from build123d import *

# Parameters (mm, degrees)
SKETCH1_R           = 1.5
BOSS_EXTRUDE1_DEPTH = 3


with BuildPart() as part:
    # Sketch1 → Boss-Extrude1 (new body)
    with BuildSketch(Plane(origin=(0, 0, 0), x_dir=(1, 0, 0), z_dir=(0, 1, 0))):
        with BuildLine():
            Line((0, 2.5), (13, 2.5))
            ThreePointArc((13, 2.5), (15.5, 0), (13, -2.5))
            Line((13, -2.5), (0, -2.5))
            ThreePointArc((0, -2.5), (-2.5, 0), (0, 2.5))
        make_face()
        with Locations(Location((0, 0, 0), (0, 0, 270))):
            Circle(SKETCH1_R, mode=Mode.SUBTRACT)
        with Locations(Location((13, 0, 0), (0, 0, 270))):
            Circle(SKETCH1_R, mode=Mode.SUBTRACT)
    extrude(amount=BOSS_EXTRUDE1_DEPTH)


solid = part.part
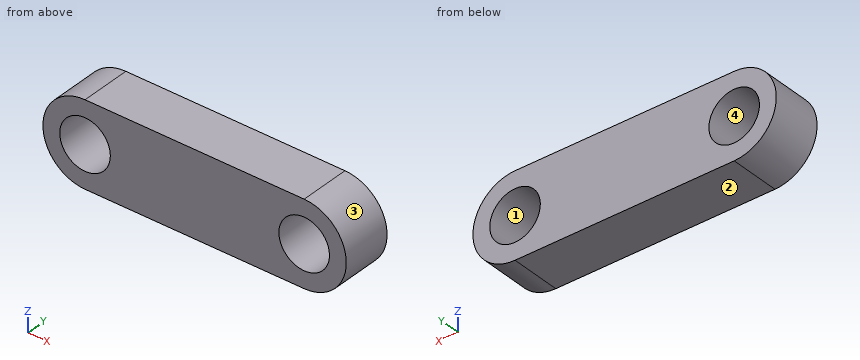
Geometry: final body of the model. Coordinates: model frame, mm. Face numbers are marked on the shaded views. Round coordinates to 2 decimals unless told otherwise and drop trailing zeros. Loops run counter-clockwise (first coordinate to the right, second up) from the corner with the lowest first, then second, coordinate; pieces in that order, holes last.
Q1. Section A-A on z = 0. Return loops of the section in (x, y), plus the area to 3 significant figures.
Q2. Section C-C on y = 0.5. Return loops of the section in (x, z), plus the area to 3 significant figures.
Q3. Section D-D on x = -0.75. Return loops of the section in (y, z).
Q4. Material intervals for L1, parallel to X at y = 2.25, z = 0; L2, parallel to X at y = 1.8, z = -1.1 (3 decimals); L3, parallel to Z at x = 12.25, y = 0.8, sorted ascending.
Q5. Pull-direction query (Z, two-part tool) for the marked faces 1, 2, 3 and 4; classes: released by +Z, released by -Z, zero draft, split by the parting line, or undercut.
Q6. Pin query (flat end, axial travel): P1, Ø1.8, axis at x = 13, z = 0, coming from the -Y side. Return the tip coordinate at first contact, or that it passes through.
Q7. Section B-B on x = 1.25. Return loops of the section in (y, z).
Evaluation:
1. outline: (-2.5, 0) - (-1.5, 0) - (-1.5, 3) - (-2.5, 3) - close; (1.5, 0) - (11.5, 0) - (11.5, 3) - (1.5, 3) - close; (14.5, 0) - (15.5, 0) - (15.5, 3) - (14.5, 3) - close
1. area: 36.0 mm2
2. outline: (0, -2.5) - (13, -2.5) arc R2.5 ccw to (13, 2.5) - (0, 2.5) arc R2.5 ccw to start; hole circle Ø3 at (0, 0); hole circle Ø3 at (13, 0)
2. area: 70.5 mm2
3. outline: (0, -2.38) - (3, -2.38) - (3, -1.3) - (0, -1.3) - close; (0, 1.3) - (3, 1.3) - (3, 2.38) - (0, 2.38) - close
4. L1: x = -2.5 to -1.5, 1.5 to 11.5, 14.5 to 15.5
4. L2: x = -2.245 to -1.02, 1.02 to 11.98, 14.02 to 15.245
4. L3: z = -2.5 to -1.3, 1.3 to 2.5
5. face 1: undercut
5. face 2: released by -Z
5. face 3: split by the parting line
5. face 4: undercut
6. P1: passes through
7. outline: (0, -2.5) - (3, -2.5) - (3, -0.83) - (0, -0.83) - close; (0, 0.83) - (3, 0.83) - (3, 2.5) - (0, 2.5) - close
